Design review of the part built by this model. Coordinates are the model's own, in mm. A direction names the side the tool comes from. Give positions to 0.01 mm unless a question says otherwise; leave off trailing zeros. Write each loop counter-clockwise with the first axis right and the second up, starting at its lowest first coordinate (ties: lowest second). Pieces come first, ordered by that corner, then holes. Notation, with made-up numbers: (16.25, 57.5) - (43.25, 57.5) arc R24 ccw to (43.25, 90.5) - close; hole circle Ø11 at (78.25, 58). An arc over 180 degrees is marked (long way). Use a Markdown table: item, result. Add a question column.
```python
from build123d import *

# Parameters (mm, degrees)
SKETCH2_W     = 0.2
SKETCH2_H     = 1.6
SKETCH2_W_2   = 0.9
SKETCH2_H_2   = 0.2
CHAMFER1_SIZE = 0.5


with BuildPart() as part:
    # Sketch1 → Revolve1 (revolve)
    with BuildSketch(Plane(origin=(0, 0, 0), x_dir=(1, 0, 0), z_dir=(0, 1, 0))):
        Polygon((0, 0), (0, -4), (21.3, -4), (21.3, -8), (151.2, -8), (151.2, -4), (171, -4), (171, 0), align=None)
    revolve(axis=Axis((-12.256689328, 0, 0), (1, 0, 0)))

    # Sketch2 → Cut-Revolve1 (revolve, cut)
    with BuildSketch(Plane(origin=(0, 0, 0), x_dir=(1, 0, 0), z_dir=(0, 1, 0))):
        with Locations((48.4, -7.2)):
            Rectangle(SKETCH2_W, SKETCH2_H)
        with Locations((143.6, -7.2)):
            Rectangle(SKETCH2_W, SKETCH2_H)
        with Locations((168.55, -3.9)):
            Rectangle(SKETCH2_W_2, SKETCH2_H_2)
        with Locations((12.45, -3.9)):
            Rectangle(SKETCH2_W_2, SKETCH2_H_2)
    revolve(axis=Axis((-6.355227553, 0, 0), (1, 0, 0)), mode=Mode.SUBTRACT)

    # Chamfer1
    chamfer1_edges = [part.edges().sort_by_distance(p)[0] for p in [
        (171, 0, -4),
        (0, 0, -4),
    ]]
    chamfer(chamfer1_edges, length=CHAMFER1_SIZE)


solid = part.part
```
(1) Tool access review of faces 1 (the face through (12.456, -0.167, -3.796)), 2 (the face through (151.2, 2, -4)), 3 (the face through (17.159, 3.905, -0.867)): name each direction out of +Z, -Z, +X, -X, +Y, -Y from which nothing blocks a thin tool from reaching the whole face with its end or side.
(2) Insertion check: pin 1 (1 mm diameter, centred on x = 76, z = -5, fed in from -Y); pin 2 (1.5 mm diameter, centred on x = 82, z = -2.5, fed in from -Y); pin 3 (1 mm diameter, centred on x = 61, y = 2, fed in from +Z). Each pin has a flat end and moves straight along its axis. Give the tip position at first contact, or say it passes through.
(3) Add section A-A (x = 96). State the section outline as (y, z) points.
(4) For line 1 along X through (y, z) = (-7.25, -1.5); line 2 along Z through (x, y) = (65, -0.5); line 3 along X through (y, z) = (-5.75, -2), list the stretches that pass through material, from the lowest coordinate up.
(5) Mouldability with a two-part tool opening along X and no side actions: class faces 4 (the face through (168.556, -0.167, -3.796)), 5 (the face through (6.33, 3.905, -0.867)), 6 (the face through (171, 0, 0)) as +X half, -X half, draft (parallel to the pull), parting line (faces both ways), or undercut.
Answers follow:
| question | item | result |
|---|---|---|
| 1 | face 1 | none |
| 1 | face 2 | +X |
| 1 | face 3 | -X |
| 2 | pin 1 | y = -6.61 |
| 2 | pin 2 | y = -7.81 |
| 2 | pin 3 | z = 7.86 |
| 3 | outline | circle Ø16 at (0, 0) |
| 4 | line 1 | 21.3 to 48.3, 48.5 to 143.5, 143.7 to 151.2 |
| 4 | line 2 | -7.98 to 7.98 |
| 4 | line 3 | 21.3 to 151.2 |
| 5 | face 4 | undercut |
| 5 | face 5 | draft |
| 5 | face 6 | +X half |
